from build123d import *

# Parameters (mm, degrees)
SKETCH1_R           = 20
SKETCH1_R_2         = 15
BOSS_EXTRUDE1_DEPTH = 26
BOSS_EXTRUDE2_START = -6
SKETCH2_R           = 30
SKETCH2_R_2         = 15
BOSS_EXTRUDE2_DEPTH = 6
FILLET1_R           = 3
CHAMFER2_SIZE       = 0.5


with BuildPart() as part:
    # Sketch1 → Boss-Extrude1 (new body)
    with BuildSketch(Plane.XY):
        with Locations(Location((0, 0, 0), (0, 0, 180))):
            Circle(SKETCH1_R)
        with Locations(Location((0, 0, 0), (0, 0, 180))):
            Circle(SKETCH1_R_2, mode=Mode.SUBTRACT)
    extrude(amount=BOSS_EXTRUDE1_DEPTH)

    # Sketch2 → Boss-Extrude2 (add)
    with BuildSketch(Plane.XY.offset(26).offset(BOSS_EXTRUDE2_START)):
        Circle(SKETCH2_R)
        with Locations(Location((0, 0, 0), (0, 0, 180))):
            Circle(SKETCH2_R_2, mode=Mode.SUBTRACT)
    extrude(amount=BOSS_EXTRUDE2_DEPTH)

    # Fillet1
    fillet1_edges = [part.edges().sort_by_distance(p)[0] for p in [
        (20, 0, 20),
    ]]
    fillet(fillet1_edges, radius=FILLET1_R)

    # Chamfer2
    chamfer2_edges = [part.edges().sort_by_distance(p)[0] for p in [
        (15, 0, 0),
        (15, 0, 26),
    ]]
    chamfer(chamfer2_edges, length=CHAMFER2_SIZE)


solid = part.part
Geometry: final body of the model. Coordinates: model frame, mm. A direction names the side the tool comes from. Coordinates: 2 decimals unless noted, no trailing zeros. Order: outer loops, then holes, each group sorted by start corner. A loop starts at its lowest first (then second) coordinate and runs counter-clockwise, first axis right, second up. Notation, with made-up numbers: (84.5, 30) - (103.5, 30) arc R15 ccw to (103.5, 36) - close; hole circle Ø7 at (71.25, -22). An arc over 180 degrees is marked (long way). Use one line per item in the form item = value.
1) Ray query, L1, parallel to Y at x = 0, z = 7; L2, parallel to Z at x = 23.5, y = -3; L3, parallel to Y at x = 11.5, z = 1.75. Return the intervals inside material, ascending.
Solutions:
L1 = -20 to -15, 15 to 20
L2 = 20 to 26
L3 = -16.36 to -9.63, 9.63 to 16.36
2) Section A-A (x = 0). Return loops of the section in (y, z), then the cut area to 3 significant figures.
Solutions:
outline = (-30, 20) - (-23, 20) arc R3 cw to (-20, 17) - (-20, 0) - (-15.5, 0) - (-15, 0.5) - (-15, 25.5) - (-15.5, 26) - (-30, 26) - close; (15, 0.5) - (15.5, 0) - (20, 0) - (20, 17) arc R3 cw to (23, 20) - (30, 20) - (30, 26) - (15.5, 26) - (15, 25.5) - close
area = 383 mm^2
3) Section D-D (z = 2). Return loops of the section in (x, y).
Solutions:
outline = circle Ø40 at (0, 0); hole circle Ø30 at (0, 0)
4) Mould query, pull axis Y, two halves, no side actions, for faces 1 (the face through (19.98, -0.88, 8.38)), 2 (the face through (13, -13, 26)), 3 (the face through (-8.06, -12.65, 12.82)). Classes: +Y half, -Y half, draft (parallel to the pull), parting line (faces both ways), or undercut.
Solutions:
face_1 = parting line
face_2 = draft
face_3 = undercut
5) Set-up query: faces 4 (the face through (-29.97, 1.32, 22.96)), 5 (the face through (15, -18, 20)). Return all of +Z, -Z, +X, -X, +Y, -Y with unobstructed straight access to the full face (end or side cutting, diameter ignored); none if empty.
Solutions:
face_4 = +Z, -Z
face_5 = -Z
6) Pin query (flat end, axial travel): pin 1 (3 mm diameter, centred on x = -14, z = 7.5, fed in from +Y); pin 2 (12 mm diameter, centred on x = -21, z = 17, fed in from -Y); pin 3 (5 mm diameter, centred on y = -13, z = 14.5, fed in from +X). Return the tip coordinate at first contact, or that it passes through.
Solutions:
pin_1 = 15.61
pin_2 = -25.5
pin_3 = 17.02
7) Section C-C (x = -25). Return loops of the section in (y, z).
Solutions:
outline = (-16.58, 20) - (16.58, 20) - (16.58, 26) - (-16.58, 26) - close
8) Section B-B (z = 21.5). Return loops of the section in (x, y).
Solutions:
outline = circle Ø60 at (0, 0); hole circle Ø30 at (0, 0)
